The model under review builds one solid part; all positions refer to its coordinate system, in mm. A direction names the side the tool comes from. Round coordinates to 2 decimals unless told otherwise and drop trailing zeros. Loops run counter-clockwise (first coordinate to the right, second up) from the corner with the lowest first, then second, coordinate; pieces in that order, holes last. Notation, with made-up numbers: M 84.5,44 L 122.5,44 A21 ccw 122.5,49 Z; hole C -25,-31 d11. An arc over 180 degrees is marked long. Return JSON: item names as keys, results as strings. Group by question number.
Q1. Consider section D-D (y = -40). State the section outline as (x, z) points, and give its area (3 significant figures).
Q2. Clearance check with flat-ended pins moving along their axes: pin 1 Ø2 at (y, z) = (5, -25) entering from -X; pin 2 Ø13 at (x, y) = (5, -0.5) entering from +Z; pin 3 Ø2.5 at (x, z) = (8.5, 5.5) entering from +Y; pin 4 Ø6.5 at (x, y) = (0, 40) entering from +Z. State where each tip first meets the part, or that it passes through.
Q3. To check wall thickness, follow line 1 along Y through (x, z) = (3.5, 4); line 2 along Y through (x, z) = (1.5, 3); line 3 along Z through (x, y) = (-2, 35). State the ranges of each line that lie inside material, in increasing order.
Q4. Consider section A-A (z = 3.5). State the section outline as (x, y) points, and give its area (3 significant figures).
Q5. Consider section C-C (x = -5.5). State the section outline as (y, z) points, and give its area (3 significant figures).
Q6. Draft analysis for pull direction X (two halves, no side actions). For faces 4 (the face through (0, -48, 8)), 5 (the face through (-23.254, 22.73, 7.888)), 6 (the face through (36.8, -2.4, 7.9)), state which applies: pulls with the +X half, pulls with the -X half, needs draft (parallel to the pull), parting line crosses it, or undercut.
Q7. Consider section B-B (y = 0). State the section outline as (x, z) points.
Q8. For faces 1 (the face through (23.254, -22.73, 7.888)), 2 (the face through (-8, 0, 8)), 3 (the face through (0, -20, 3)), list the 3-axis set-ups (+Z, -Z, +X, -X, +Y, -Y) from which the entire face can be reached by the end or side of a thin tool; tool diameter is ignored.
from build123d import *

# Parameters (mm, degrees)
FLANGE_PLATE_SKETCH_R    = 4
FLANGE_PLATE_SKETCH_R_2  = 32
FLANGE_PLATE_4_LUG_DEPTH = 16
FRONT_RECESS_32_SKETCH_R = 32
FRONT_RECESS_32_DEPTH    = 10
ARC_SLOTS_DEPTH          = 6
FRONT_HUB_14_SKETCH_R    = 14
FRONT_HUB_14_DEPTH       = 10
REAR_START               = 34
REAR_HUB_14_SKETCH_R     = 14
REAR_HUB_14_DEPTH        = 34
KEYED_BORE_8_DEPTH       = 16


with BuildPart() as part:
    # Flange Plate Sketch → Flange Plate 4-Lug (new body)
    # profile 1 of 2: a face of its own
    with BuildSketch(Plane.XY):
        with BuildLine():
            ThreePointArc((-6.940896525, -43.977933562), (-22.991424972, -22.991424972), (-43.977933562, -6.940896525))
            ThreePointArc((-43.977933562, -6.940896525), (-48, 0), (-43.977933562, 6.940896525))
            ThreePointArc((-43.977933562, 6.940896525), (-22.991424972, 22.991424972), (-6.940896525, 43.977933562))
            ThreePointArc((-6.940896525, 43.977933562), (0, 48), (6.940896525, 43.977933562))
            ThreePointArc((6.940896525, 43.977933562), (22.991424972, 22.991424972), (43.977933562, 6.940896525))
            ThreePointArc((43.977933562, 6.940896525), (48, 0), (43.977933562, -6.940896525))
            ThreePointArc((43.977933562, -6.940896525), (22.991424972, -22.991424972), (6.940896525, -43.977933562))
            ThreePointArc((6.940896525, -43.977933562), (0, -48), (-6.940896525, -43.977933562))
        make_face()
        with Locations((0, -40)):
            Circle(FLANGE_PLATE_SKETCH_R, mode=Mode.SUBTRACT)
        with Locations((-40, 0)):
            Circle(FLANGE_PLATE_SKETCH_R, mode=Mode.SUBTRACT)
        with Locations((40, 0)):
            Circle(FLANGE_PLATE_SKETCH_R, mode=Mode.SUBTRACT)
        with Locations((0, 40)):
            Circle(FLANGE_PLATE_SKETCH_R, mode=Mode.SUBTRACT)
        Circle(FLANGE_PLATE_SKETCH_R_2, mode=Mode.SUBTRACT)
    # profile 2 of 2: a face of its own
    with BuildSketch(Plane.XY):
        Circle(FLANGE_PLATE_SKETCH_R_2)
    extrude(amount=FLANGE_PLATE_4_LUG_DEPTH)

    # Front Recess Ø32 Sketch → Front Recess Ø32 (cut)
    with BuildSketch(Plane.XY.offset(16)):
        Circle(FRONT_RECESS_32_SKETCH_R)
    extrude(amount=-FRONT_RECESS_32_DEPTH, mode=Mode.SUBTRACT)

    # Arc Slots Sketch → Arc Slots (cut)
    with BuildSketch(Plane.XY.offset(6)):
        with BuildLine():
            ThreePointArc((-18.384776311, -18.384776311), (0, -26), (18.384776311, -18.384776311))
            ThreePointArc((18.384776311, -18.384776311), (18.384776311, -14.142135624), (14.142135624, -14.142135624))
            ThreePointArc((14.142135624, -14.142135624), (0, -20), (-14.142135624, -14.142135624))
            ThreePointArc((-14.142135624, -14.142135624), (-18.384776311, -14.142135624), (-18.384776311, -18.384776311))
        make_face()
        with BuildLine():
            ThreePointArc((14.142135624, 14.142135624), (0, 20), (-14.142135624, 14.142135624))
            ThreePointArc((-14.142135624, 14.142135624), (-18.384776311, 14.142135624), (-18.384776311, 18.384776311))
            ThreePointArc((-18.384776311, 18.384776311), (0, 26), (18.384776311, 18.384776311))
            ThreePointArc((18.384776311, 18.384776311), (18.384776311, 14.142135624), (14.142135624, 14.142135624))
        make_face()
    extrude(amount=-ARC_SLOTS_DEPTH, mode=Mode.SUBTRACT)

    # Front Hub Ø14 Sketch → Front Hub Ø14 (add)
    with BuildSketch(Plane.XY.offset(6)):
        Circle(FRONT_HUB_14_SKETCH_R)
    extrude(amount=FRONT_HUB_14_DEPTH)

    # Rear Hub Ø14 Sketch → Rear Hub Ø14 (add)
    with BuildSketch(Plane(origin=(0, 0, 0), x_dir=(-1, 0, 0), z_dir=(0, 0, -1)).offset(REAR_START)):
        with Locations(Location((0, 0, 0), (0, 0, 180))):
            Circle(REAR_HUB_14_SKETCH_R)
    extrude(amount=-REAR_HUB_14_DEPTH)

    # Keyed Bore Ø8 Sketch → Keyed Bore Ø8 (cut)
    with BuildSketch(Plane.XY.offset(16)):
        with BuildLine():
            Line((9.85, 0), (9.85, 1.99))
            Line((9.85, 1.99), (7.748541798, 1.99))
            ThreePointArc((7.748541798, 1.99), (-8, 0), (7.748541798, -1.99))
            Line((7.748541798, -1.99), (9.85, -1.99))
            Line((9.85, -1.99), (9.85, 0))
        make_face()
    extrude(amount=-KEYED_BORE_8_DEPTH, mode=Mode.SUBTRACT)


solid = part.part
Values:
{
 "1": {"outline": "M -9.35,0 L -4,0 L -4,16 L -9.35,16 Z; M 4,0 L 9.35,0 L 9.35,16 L 4,16 Z", "area": "171 mm2"},
 "2": {"pin 1": "stops at x = -13.42", "pin 2": "stops at z = 16", "pin 3": "stops at y = 43.44", "pin 4": "passes through"},
 "3": {"line 1": "y = -47.19 to -41.94, -38.06 to -25.76, -19.69 to -7.19, 7.19 to 19.69, 25.76 to 38.06, 41.94 to 47.19", "line 2": "y = -47.86 to -43.71, -36.29 to -25.96, -19.94 to -7.86, 7.86 to 19.94, 25.96 to 36.29, 43.71 to 47.86", "line 3": "z = 0 to 16"},
 "4": {"outline": "M -43.98,-6.94 A100 cw -6.94,-43.98 A8 ccw 6.94,-43.98 A100 cw 43.98,-6.94 A8 ccw 43.98,6.94 A100 cw 6.94,43.98 A8 ccw -6.94,43.98 A100 cw -43.98,6.94 A8 ccw Z; hole C -40,0 d8; hole M -18.38,-18.38 A26 ccw 18.38,-18.38 A3 ccw 14.14,-14.14 A20 cw -14.14,-14.14 A3 ccw Z; hole M -18.38,18.38 A3 ccw -14.14,14.14 A20 cw 14.14,14.14 A3 ccw 18.38,18.38 A26 ccw Z; hole C 0,-40 d8; hole C 0,40 d8; hole M 7.75,-1.99 L 9.85,-1.99 L 9.85,1.99 L 7.75,1.99 A8 ccw long Z; hole C 40,0 d8", "area": "3,760 mm2"},
 "5": {"outline": "M -45.81,0 L -25.41,0 L -25.41,6 L -31.52,6 L -31.52,16 L -45.81,16 Z; M -19.23,0 L -12.87,0 L -12.87,-34 L 12.87,-34 L 12.87,0 L 19.23,0 L 19.23,6 L 12.87,6 L 12.87,16 L 5.81,16 L 5.81,0 L -5.81,0 L -5.81,16 L -12.87,16 L -12.87,6 L -19.23,6 Z; M 25.41,0 L 45.81,0 L 45.81,16 L 31.52,16 L 31.52,6 L 25.41,6 Z", "area": "1,710 mm2"},
 "6": {"face 4": "parting line crosses it", "face 5": "pulls with the -X half", "face 6": "undercut"},
 "7": {"outline": "M -48,0 L -44,0 L -44,16 L -48,16 Z; M -36,0 L -14,0 L -14,-34 L 14,-34 L 14,0 L 36,0 L 36,16 L 32,16 L 32,6 L 14,6 L 14,16 L 9.85,16 L 9.85,0 L -8,0 L -8,16 L -14,16 L -14,6 L -32,6 L -32,16 L -36,16 Z; M 44,0 L 48,0 L 48,16 L 44,16 Z"},
 "8": {"face 1": "+Z, -Z, +X, -Y", "face 2": "+Z", "face 3": "+Z, -Z"}
}
